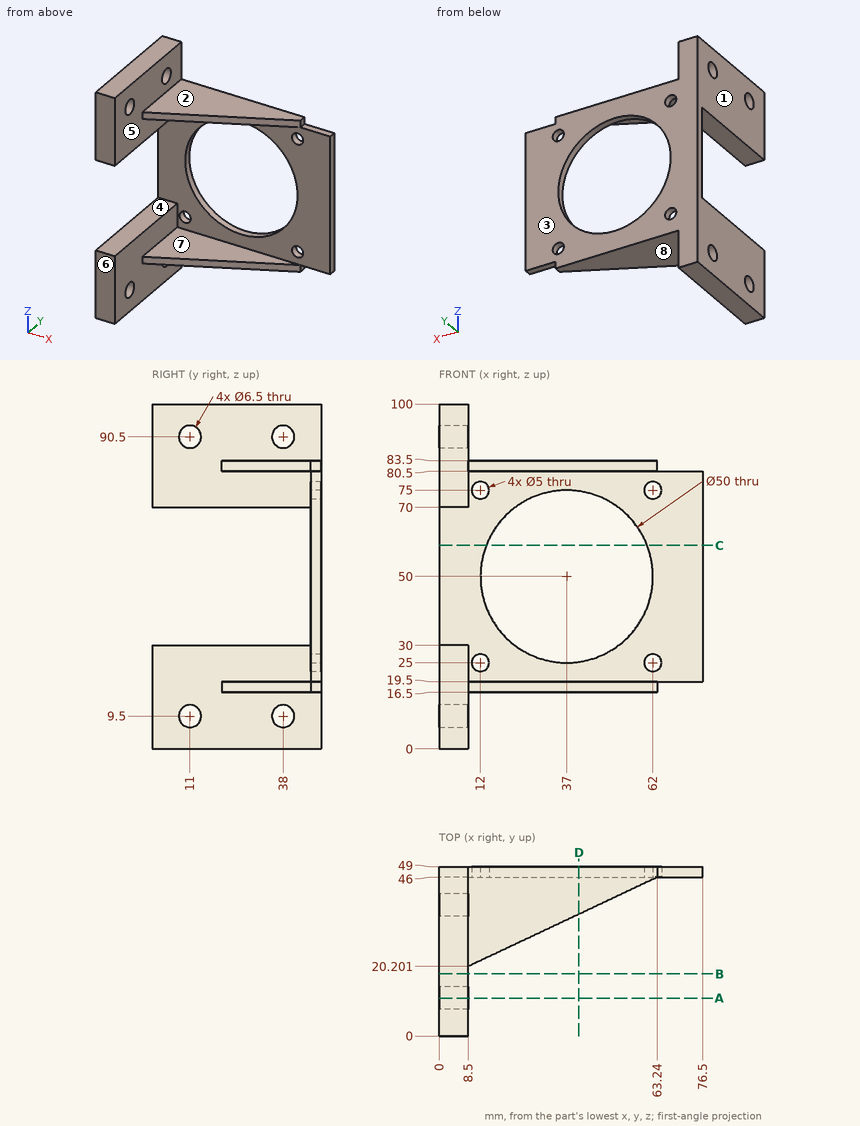
Here's the drawing with two shaded views (mm, measured from the low corner). I have some questions. A direction names the side the tool comes from. Round coordinates to 2 decimals unless told otherwise and drop trailing zeros. Order: outer loops, then holes, each group sorted by start corner. A loop starts at its lowest first (then second) coordinate and runs counter-clockwise, first axis right, second up. Notation, with made-up numbers: M 48,-15.75 L 57,-15.75 A29 cw 57,12.25 Z; hole C 8.25,57.25 d8. An arc over 180 degrees is marked long. Use CSV: the item, a comma, the result in double quotes.
1) If we mould it in two halves opening along Z, with no side actions, what happens to the marked faces 6, 7 and 8? For each: pulls with the +Z half, pulls with the -Z half, needs draft (parallel to the pull), parting line crosses it, or undercut.
Taken from the geometry:
face 6,"needs draft"
face 7,"undercut"
face 8,"pulls with the -Z half"
2) I'm going to push flat-ended pins straight in: P1, Ø2, axis at x = 26, z = 16, coming from the +Y side; P2, Ø4, axis at x = 25, y = 35, coming from the +Z side; P3, Ø2, axis at x = 16.5, z = 22, coming from the -Y side; P4, Ø8.5, axis at y = 38, z = 90.5, coming from the +X side. Where does each tip first touch, or does it pass through?
Taken from the geometry:
P1,"y = 49"
P2,"z = 83.5"
P3,"y = 46"
P4,"x = 8.5"
3) I want a section at A-A (y = 11). List the corners of the cut face in (x, z) for me.
Taken from the geometry:
outline,"M 0,0 L 8.5,0 L 8.5,6.25 L 0,6.25 Z; M 0,12.75 L 8.5,12.75 L 8.5,30 L 0,30 Z; M 0,70 L 8.5,70 L 8.5,87.25 L 0,87.25 Z; M 0,93.75 L 8.5,93.75 L 8.5,100 L 0,100 Z"
4) I want a section at C-C (z = 59). List the corners of the cut face in (x, y) for me.
Taken from the geometry:
outline,"M 0,46 L 13.68,46 L 13.68,49 L 0,49 Z; M 60.32,46 L 76.5,46 L 76.5,49 L 60.32,49 Z"
5) I want a section at D-D (x = 40.5). List the corners of the cut face in (y, z) for me.
Taken from the geometry:
outline,"M 35.28,16.5 L 49,16.5 L 49,25.25 L 46,25.25 L 46,19.5 L 35.28,19.5 Z; M 35.28,80.5 L 46,80.5 L 46,74.75 L 49,74.75 L 49,83.5 L 35.28,83.5 Z"
6) I want a section at B-B (y = 18). List the corners of the cut face in (x, z) for me, then the cut area to 3 significant figures.
Taken from the geometry:
outline,"M 0,0 L 8.5,0 L 8.5,30 L 0,30 Z; M 0,70 L 8.5,70 L 8.5,100 L 0,100 Z"
area,"510 mm^2"
7) I need wall thicknesses on line 1 along Y through (x, z) = (2.5, 90.5); line 2 along Z through (x, y) = (20.5, 33); line 3 along Z through (x, y) = (7, 4). Which ranges of each line are inside material? Lowest first, please. Write a range as [from, to].
Taken from the geometry:
line 1,"[0, 7.75], [14.25, 34.75], [41.25, 49]"
line 2,"[16.5, 19.5], [80.5, 83.5]"
line 3,"[0, 30], [70, 100]"
8) On a 3-axis mill with a long thin cutter (end or side, diameter ignored), from which of +Z, -Z, +X, -X, +Y, -Y can I reach the whole of each face in a straight line? I mean the marked faces 1, 2, 3, 4 and 5. Say none if no direction works.
Taken from the geometry:
face 1,"+Z, -Z, -X, +Y, -Y"
face 2,"+Z, +X, +Y, -Y"
face 3,"+Z, -Z, +X, -X, +Y"
face 4,"+X, -X, -Y"
face 5,"+X, -Y"
